The listing builds one solid part. Answer for the finished solid, in the listing's coordinates (mm). A direction names the side the tool comes from. Give positions to 0.01 mm unless a question says otherwise; leave off trailing zeros. Loops run counter-clockwise (first coordinate to the right, second up) from the corner with the lowest first, then second, coordinate; pieces in that order, holes last.
Item 1: A tool of negligible diameter and unlimited length cuts with its end or side. For faces 1 (the face through (14, 6, 64.4)), 2 (the face through (19, 1, 0)), 3 (the face through (-11, 17, 58.4)), from which of +Z, -Z, +X, -X, +Y, -Y can it reach the whole face along a straight path? Write none if from no direction.
Item 2: The mould has two halves that part along Z. Classify faces 4 (the face through (0.8, 38.7, 7)), 5 (the face through (-4, 19, 88.4)), 6 (the face through (-4.336, -19.524, 37.258)), 7 (the face through (7.023, -13.502, 2.812)): pulls with the +Z half, pulls with the -Z half, needs draft (parallel to the pull), parting line crosses it, or undercut.
Item 3: Each of these flat-tipped pins is pushed along its axis until it touches: pin 1 Ø20 at (x, y) = (0, -32.5) entering from -Z; pin 2 Ø1 at (x, y) = (6, -33.5) entering from +Z; pin 3 Ø2 at (y, z) = (-14.5, 78.5) entering from -X; pin 4 Ø6 at (x, z) = (-23, 62.5) entering from -Y. Where does it stop, or does it pass through?
Item 4: Consider line 1 along Y through (x, z) = (0, 11.5); line 2 along Y through (x, z) = (0, 72); line 3 along Z through (x, y) = (21, -12). Determine where each line is inside the solid, lowest interval first.
Item 5: Section C-C, the plane z = 41.5 is taken. Give the vertices of the cut face in (x, y), and give its area (3 significant figures).
Item 6: Section A-A, the plane y = 0 is taken. Give the number of separate pieces and of enclosed holes in the cut face, and give its area (3 significant figures).
from build123d import *

# Parameters (mm, degrees)
FLANGE_PROFILE_SKETCH_R       = 45
FLANGE_PROFILE_SKETCH_R_2     = 15
FLANGE_90_DEPTH               = 14.2
FLANGE_HOLES_SKETCH_R         = 6.25
FLANGE_HOLES_4X_12_5_DEPTH    = 66.204601065
FLANGE_CHAMFER_SIZE           = 3
FLANGE_CHAMFER_SIZE2          = 3.5
NECK_PROFILE_SKETCH_R         = 20
NECK_PROFILE_SKETCH_R_2       = 15
NECK_40_DEPTH                 = 44.2
FLANGE_EDGE_FILLET_R2_5_R     = 2.5
COLLAR_PROFILE_SKETCH_R       = 25
COLLAR_PROFILE_SKETCH_R_2     = 15
COLLAR_50_DEPTH               = 6
END_SLEEVE_PROFILE_SKETCH_R   = 25
END_SLEEVE_PROFILE_SKETCH_R_2 = 19
END_SLEEVE_50_BORE_38_DEPTH   = 24
NECK_ROOT_FILLET_R2_5_R       = 2.5


with BuildPart() as part:
    # Flange Profile Sketch → Flange Ø90 (new body)
    with BuildSketch(Plane.XY):
        Circle(FLANGE_PROFILE_SKETCH_R)
        Circle(FLANGE_PROFILE_SKETCH_R_2, mode=Mode.SUBTRACT)
    extrude(amount=FLANGE_90_DEPTH)

    # Flange Holes Sketch → Flange Holes 4xØ12.5 (cut, through all)
    with BuildSketch(Plane(origin=(0, 0, 0), x_dir=(-1, 0, 0), z_dir=(0, 0, -1))):
        with Locations((-32.5, 0)):
            Circle(FLANGE_HOLES_SKETCH_R)
        with Locations((32.5, 0)):
            Circle(FLANGE_HOLES_SKETCH_R)
        with Locations((0, -32.5)):
            Circle(FLANGE_HOLES_SKETCH_R)
        with Locations((0, 32.5)):
            Circle(FLANGE_HOLES_SKETCH_R)
    extrude(amount=-FLANGE_HOLES_4X_12_5_DEPTH, mode=Mode.SUBTRACT)

    # Flange Chamfer
    flange_chamfer_edges = [part.edges().sort_by_distance(p)[0] for p in [
        (-15, 0, 0),
    ]]
    flange_chamfer_side = [part.faces().sort_by_distance(p)[0] for p in [
        (-15, 0, 7.1),
    ]]
    chamfer(flange_chamfer_edges, length=FLANGE_CHAMFER_SIZE, length2=FLANGE_CHAMFER_SIZE2, reference=flange_chamfer_side[0])

    # Neck Profile Sketch → Neck Ø40 (add)
    with BuildSketch(Plane.XY.offset(14.2)):
        Circle(NECK_PROFILE_SKETCH_R)
        Circle(NECK_PROFILE_SKETCH_R_2, mode=Mode.SUBTRACT)
    extrude(amount=NECK_40_DEPTH)

    # Flange Edge Fillet R2.5
    flange_edge_fillet_r2_5_edges = [part.edges().sort_by_distance(p)[0] for p in [
        (-45, 0, 14.2),
    ]]
    fillet(flange_edge_fillet_r2_5_edges, radius=FLANGE_EDGE_FILLET_R2_5_R)

    # Collar Profile Sketch → Collar Ø50 (add)
    with BuildSketch(Plane.XY.offset(58.4)):
        Circle(COLLAR_PROFILE_SKETCH_R)
        Circle(COLLAR_PROFILE_SKETCH_R_2, mode=Mode.SUBTRACT)
    extrude(amount=COLLAR_50_DEPTH)

    # End Sleeve Profile Sketch → End Sleeve Ø50 Bore Ø38 (add)
    with BuildSketch(Plane.XY.offset(64.4)):
        Circle(END_SLEEVE_PROFILE_SKETCH_R)
        Circle(END_SLEEVE_PROFILE_SKETCH_R_2, mode=Mode.SUBTRACT)
    extrude(amount=END_SLEEVE_50_BORE_38_DEPTH)

    # Neck Root Fillet R2.5
    neck_root_fillet_r2_5_edges = [part.edges().sort_by_distance(p)[0] for p in [
        (-20, 0, 14.2),
    ]]
    fillet(neck_root_fillet_r2_5_edges, radius=NECK_ROOT_FILLET_R2_5_R)


solid = part.part
Worked answers:
1. face 1: +Z
1. face 2: -Z, +X, -X, +Y, -Y
1. face 3: none
2. face 4: needs draft
2. face 5: pulls with the +Z half
2. face 6: undercut
2. face 7: pulls with the -Z half
3. pin 1: stops at z = 0
3. pin 2: stops at z = 14.2
3. pin 3: stops at x = -21.04
3. pin 4: stops at y = -15
4. line 1: y = -45 to -38.75, -26.25 to -15, 15 to 26.25, 38.75 to 45
4. line 2: y = -25 to -19, 19 to 25
4. line 3: z = 0 to 14.2, 58.4 to 88.4
5. outline: circle Ø40 at (0, 0); hole circle Ø30 at (0, 0)
5. area: 550 mm2
6. separate pieces: 4
6. enclosed holes: 0
6. area: 1,340 mm2
